Geometry check sheet. Reference: the model listing, model coordinates, mm. A direction names the side the tool comes from. Give positions to 0.01 mm unless a question says otherwise; leave off trailing zeros. Loops run counter-clockwise (first coordinate to the right, second up) from the corner with the lowest first, then second, coordinate; pieces in that order, holes last. Notation, with made-up numbers: (6.25, 16.25) -> (11.25, 16.25) arc R22 cw to (11.25, 40.25) -> close; hole circle Ø4 at (7, 78). An arc over 180 degrees is marked (long way). Write each question's results on one line, items separated by ' | '. Start each with the question number.
1) Draft check along X on faces 5 (the face through (-101.9, 59, 25)), 6 (the face through (-7.859, 5, -1)), 7 (the face through (35, 42, -1)). Enter one of: pulls with the +X half, pulls with the -X half, needs draft (parallel to the pull), parting line crosses it, or undercut.
2) Depth check by flat-ended pin: pin 1 (1.5 mm diameter, centred on x = -59.5, z = -19, fed in from +Y); pin 2 (12 mm diameter, centred on y = 156, z = 17.5, fed in from -X); pin 3 (10 mm diameter, centred on x = -55, y = 161.5, fed in from +Z). Enter the tip coordinate at first touch or a pass-through.
3) Sectioned sample at D-D on x = 11. Record the cut outline in (y, z).
4) Sectioned sample at A-A on y = 75. Record the cut outline in (x, z), then the cut area to 3 significant figures.
5) Scan lines: line 1 (Z direction, x = 66, y = 43); line 2 (Z direction, x = -47, y = 53); line 3 (Y direction, x = 65, z = 86). Record each from-to range of solid material in increasing order. Write a range as from..to.
6) Sectioned sample at C-C on z = -65.5. Record the cut outline in (x, y).
7) Sectioned sample at B-B on x = -107. Record the cut outline in (y, z).
8) Set-up check for faces 1 (the face through (-39, 54, -60)), 2 (the face through (30, 205, 70)), 3 (the face through (30, 205, -70)), 4 (the face through (68, 48, 73)): record each of +Z, -Z, +X, -X, +Y, -Y from which the full face is reachable in a straight line by a thin tool's end or side.
```python
from build123d import *
from build123d.topology import SkipClean

# Parameters (mm, degrees)
BASE_PLATE_PROFILE_R       = 12.5
BASE_PLATE_DEPTH           = 42
UPRIGHT_PROFILE_W          = 30
UPRIGHT_PROFILE_H          = 120
UPRIGHT_WEB_DEPTH          = 166
UPPER_BLOCK_DEPTH          = 10
UPPER_BLOCK_DEPTH_BACK     = 130
UPPER_BLOCK_PROFILE_R      = 57.5
UPPER_BLOCK_PROFILE_R_2    = 37.5
UPPER_BLOCK_TRIM_CUT_DEPTH = 130
HOUSING_PROFILE_R          = 37.5
HOUSING_PROFILE_R_2        = 22.5
HOUSING_DEPTH              = 13
SIDE_BOSS_DEPTH            = 12
SIDE_BOSS_DEPTH_BACK       = 39
SIDE_BOSS_PROFILE_R        = 37.280115622
BORE_45_PROFILE_R          = 22.5
BORE_45_DEPTH              = 203
MOUNTING_PADS_PROFILE_R    = 30
MOUNTING_PADS_PROFILE_R_2  = 12.5
MOUNTING_PADS_DEPTH        = 6
MOUNTING_HOLES_DEPTH       = 85
MOUNTING_HOLES_DEPTH_BACK  = 317
MOUNTING_HOLES_PROFILE_W   = 111
MOUNTING_HOLES_PROFILE_H   = 9.419031608


with BuildPart() as part:
    # Base Plate Profile → Base Plate (new body)
    with BuildSketch(Plane(origin=(0, 0, 0), x_dir=(1, 0, 0), z_dir=(0, 1, 0))):
        with BuildLine():
            Line((-65.358744395, 60), (31.141255605, 60))
            ThreePointArc((31.141255605, 60), (67.141255605, 96), (103.141255605, 60))
            Line((103.141255605, 60), (103.141255605, -60))
            ThreePointArc((103.141255605, -60), (67.141255605, -96), (31.141255605, -60))
            Line((31.141255605, -60), (-65.358744395, -60))
            Line((-65.358744395, -60), (-65.358744395, 60))
        make_face()
        with Locations(Location((67.141255605, -60, 0), (0, 0, 90))):
            Circle(BASE_PLATE_PROFILE_R, mode=Mode.SUBTRACT)
        with Locations(Location((67.141255605, 60, 0), (0, 0, 90))):
            Circle(BASE_PLATE_PROFILE_R, mode=Mode.SUBTRACT)
    extrude(amount=BASE_PLATE_DEPTH)

    # Upright Profile → Upright Web (add)
    with BuildSketch(Plane(origin=(0, 42, 0), x_dir=(1, 0, 0), z_dir=(0, 1, 0))):
        with Locations((-50.358744395, 0)):
            Rectangle(UPRIGHT_PROFILE_W, UPRIGHT_PROFILE_H)
    extrude(amount=UPRIGHT_WEB_DEPTH)

    # Upper Block Profile → Upper Block (add, two sides: drawn at the far end of the back side and taken through both)
    with BuildSketch(Plane.XY.offset(60).offset(-UPPER_BLOCK_DEPTH_BACK)):
        with Locations((-7.975662641, 204.33504045)):
            Circle(UPPER_BLOCK_PROFILE_R)
        with Locations((-7.975662641, 204.33504045)):
            Circle(UPPER_BLOCK_PROFILE_R_2, mode=Mode.SUBTRACT)
    extrude(amount=UPPER_BLOCK_DEPTH + UPPER_BLOCK_DEPTH_BACK)

    # Upper Block Trim Profile → Upper Block Trim Cut (cut)
    with SkipClean():  # the faces are left unmerged after this step: merging them gives an invalid solid
        with BuildSketch(Plane.XY.offset(60)):
            with BuildLine():
                Line((-45.296140552, 208), (-35.358744395, 208))
                Line((-35.358744395, 208), (-35.358744395, 178.714407481))
                ThreePointArc((-35.358744395, 178.714407481), (-43.486916359, 192.285108524), (-45.296140552, 208))
            make_face()
        extrude(amount=-UPPER_BLOCK_TRIM_CUT_DEPTH, mode=Mode.SUBTRACT)

    # Housing Profile → Housing (add, symmetric)
    # profile 1 of 2: a face of its own
    with BuildSketch(Plane.XY):
        with BuildLine():
            ThreePointArc((-80.475662641, 75), (-99.448917842, 42.396170054), (-137.169514756, 42.784382033))
            Line((-137.169514756, 42.784382033), (-65.358744395, 0))
            Line((-65.358744395, 0), (-65.358744395, 200.670080899))
            ThreePointArc((-65.358744395, 200.670080899), (-63.521325311, 219.198733078), (-55.859494126, 236.168806836))
            Line((-55.859494126, 236.168806836), (-149.204248392, 95.761151991))
            ThreePointArc((-149.204248392, 95.761151991), (-107.131815668, 110.897924492), (-80.475662641, 75))
        make_face()
    # profile 2 of 2: a face of its own
    with BuildSketch(Plane.XY):
        with Locations((-117.975662641, 75)):
            Circle(HOUSING_PROFILE_R)
        with Locations(Location((-117.975662641, 75, 0), (0, 0, 180))):
            Circle(HOUSING_PROFILE_R_2, mode=Mode.SUBTRACT)
    extrude(amount=HOUSING_DEPTH, both=True)

    # Side Boss Profile → Side Boss (add, two sides: drawn at the far end of the back side and taken through both)
    with BuildSketch(Plane.XY.offset(13).offset(-SIDE_BOSS_DEPTH_BACK)):
        with Locations((-117.975662641, 75)):
            Circle(SIDE_BOSS_PROFILE_R)
    extrude(amount=SIDE_BOSS_DEPTH + SIDE_BOSS_DEPTH_BACK)

    # Bore Ø45 Profile → Bore Ø45 (cut)
    with BuildSketch(Plane.XY.offset(25)):
        with Locations((-117.975662641, 75)):
            Circle(BORE_45_PROFILE_R)
    extrude(amount=-BORE_45_DEPTH, mode=Mode.SUBTRACT)

    # Mounting Pads Profile → Mounting Pads (add)
    # profile 1 of 2: a face of its own
    with BuildSketch(Plane(origin=(0, 42, 0), x_dir=(1, 0, 0), z_dir=(0, 1, 0))):
        with Locations(Location((67.141255605, -60, 0), (0, 0, 270))):
            Circle(MOUNTING_PADS_PROFILE_R)
        with Locations(Location((67.141255605, -60, 0), (0, 0, 90))):
            Circle(MOUNTING_PADS_PROFILE_R_2, mode=Mode.SUBTRACT)
    # profile 2 of 2: a face of its own
    with BuildSketch(Plane(origin=(0, 42, 0), x_dir=(1, 0, 0), z_dir=(0, 1, 0))):
        with Locations(Location((67.141255605, 60, 0), (0, 0, 270))):
            Circle(MOUNTING_PADS_PROFILE_R)
        with Locations(Location((67.141255605, 60, 0), (0, 0, 90))):
            Circle(MOUNTING_PADS_PROFILE_R_2, mode=Mode.SUBTRACT)
    extrude(amount=MOUNTING_PADS_DEPTH)

    # Mounting Holes Profile → Mounting Holes (cut, two sides: drawn at the far end of the back side and taken through both)
    with BuildSketch(Plane.XY.offset(60).offset(-MOUNTING_HOLES_DEPTH_BACK)):
        with Locations((47.641255605, 4.709515804)):
            Rectangle(MOUNTING_HOLES_PROFILE_W, MOUNTING_HOLES_PROFILE_H)
    extrude(amount=MOUNTING_HOLES_DEPTH + MOUNTING_HOLES_DEPTH_BACK, mode=Mode.SUBTRACT)


solid = part.part
```
Result:
1) face 5: needs draft | face 6: pulls with the +X half | face 7: undercut
2) pin 1: y = 231.32 | pin 2: x = -111.8 | pin 3: z = 60
3) outline: (9.42, -60) -> (42, -60) -> (42, 60) -> (9.42, 60) -> close; (150.06, -70) -> (171.99, -70) -> (171.99, 70) -> (150.06, 70) -> close; (236.68, -70) -> (258.61, -70) -> (258.61, 70) -> (236.68, 70) -> close
4) outline: (-155.48, -13) -> (-155.26, -13) -> (-155.26, -26) -> (-140.48, -26) -> (-140.48, 25) -> (-155.26, 25) -> (-155.26, 13) -> (-155.48, 13) -> close; (-95.48, -26) -> (-80.7, -26) -> (-80.7, -13) -> (-65.36, -13) -> (-65.36, -60) -> (-35.36, -60) -> (-35.36, 60) -> (-65.36, 60) -> (-65.36, 13) -> (-80.7, 13) -> (-80.7, 25) -> (-95.48, 25) -> close | area: 5,510 mm^2
5) line 1: -89.98..-72.45, -47.55..-30.02, 30.02..47.55, 72.45..89.98 | line 2: -60..60 | line 3: 9.42..48
6) outline: circle Ø115 at (-7.98, 204.34); (31.56, 9.42) -> (55.92, 9.42) -> (55.92, 48) -> (37.65, 48) -> (37.65, 42) -> (31.56, 42) -> close; (78.37, 9.42) -> (102.72, 9.42) -> (102.72, 42) -> (96.63, 42) -> (96.63, 48) -> (78.37, 48) -> close; hole circle Ø75 at (-7.98, 204.34)
7) outline: (24.81, -13) -> (39.37, -13) -> (39.37, -26) -> (55.36, -26) -> (55.36, 25) -> (39.37, 25) -> (39.37, 13) -> (24.81, 13) -> close; (94.64, -26) -> (110.63, -26) -> (110.63, -13) -> (159.24, -13) -> (159.24, 13) -> (110.63, 13) -> (110.63, 25) -> (94.64, 25) -> close
8) face 1: -Z, -X, -Y | face 2: +Z, +X, -X, +Y | face 3: -Z, +X, -X, +Y | face 4: +Z, -Z, +X
